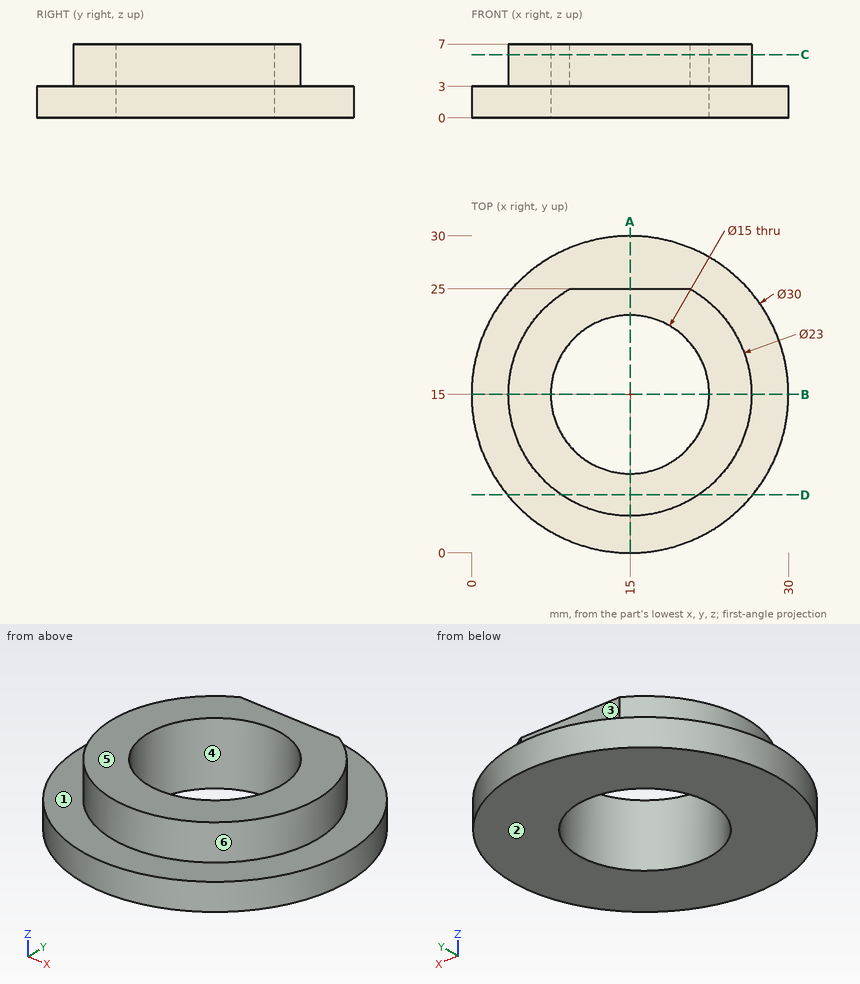
Check sheet for the drawn part. Datum: minimum x, y, z corner. Units: mm. A direction names the side the tool comes from. Coordinates: 2 decimals unless noted, no trailing zeros. Write each loop counter-clockwise with the first axis right and the second up, starting at its lowest first coordinate (ties: lowest second). Pieces come first, ordered by that corner, then holes. Notation, with made-up numbers: M -22,46 L 19,46 A16 cw 19,51 Z; hole C 58,-35 d1. An arc over 180 degrees is marked long. Use a Markdown table: item, result.
Q1. Thickness scan on line 1 (X direction, y = 17, z = 2); line 2 (Z direction, x = 22.5, y = 6.25); line 3 (X direction, y = 12.5, z = 6). Record the ranges inside material, lowest first.
Reply:
| item | result |
|---|---|
| line 1 | x = 0.13 to 7.77, 22.23 to 29.87 |
| line 2 | z = 0 to 3 |
| line 3 | x = 3.78 to 7.93, 22.07 to 26.22 |
Q2. Draft check along X on the marked faces 4, 5 and 6. Enter one of: +X half, -X half, draft (parallel to the pull), parting line (faces both ways), or undercut.
Reply:
| item | result |
|---|---|
| face 4 | undercut |
| face 5 | draft |
| face 6 | parting line |
Q3. Set-up check for the marked faces 1, 2 and 3: record each of +Z, -Z, +X, -X, +Y, -Y from which the full face is reachable in a straight line by a thin tool's end or side.
Reply:
| item | result |
|---|---|
| face 1 | +Z |
| face 2 | -Z, +X, -X, +Y, -Y |
| face 3 | +Z, +X, -X, +Y |
Q4. Go/stop test with flat-tipped pins: P1, Ø3, axis at x = 6.5, z = 2, coming from the -Y side; P2, Ø2, axis at y = 7, z = 5, coming from the -X side; P3, Ø2, axis at y = 22.5, z = 1, coming from the +X side. Record where each tip stops, or that it passes through.
Reply:
| item | result |
|---|---|
| P1 | stops at y = 1.73 |
| P2 | stops at x = 5.88 |
| P3 | stops at x = 28.52 |
Q5. Sectioned sample at D-D, the plane y = 5.5. Record the boundary of the cut face in (x, z).
Reply:
| item | result |
|---|---|
| outline | M 3.39,0 L 26.61,0 L 26.61,3 L 21.48,3 L 21.48,7 L 8.52,7 L 8.52,3 L 3.39,3 Z |
Q6. Sectioned sample at C-C, the plane z = 6. Record the boundary of the cut face in (x, y), plus the area to 3 significant figures.
Reply:
| item | result |
|---|---|
| outline | M 9.32,25 A11.5 ccw long 20.68,25 Z; hole C 15,15 d15 |
| area | 227 mm² |
Q7. Sectioned sample at B-B, the plane y = 15. Record the boundary of the cut face in (x, z), plus the area to 3 significant figures.
Reply:
| item | result |
|---|---|
| outline | M 0,0 L 7.5,0 L 7.5,7 L 3.5,7 L 3.5,3 L 0,3 Z; M 22.5,0 L 30,0 L 30,3 L 26.5,3 L 26.5,7 L 22.5,7 Z |
| area | 77.0 mm² |
Q8. Sectioned sample at A-A, the plane x = 15. Record the boundary of the cut face in (y, z), plus the area to 3 significant figures.
Reply:
| item | result |
|---|---|
| outline | M 0,0 L 7.5,0 L 7.5,7 L 3.5,7 L 3.5,3 L 0,3 Z; M 22.5,0 L 30,0 L 30,3 L 25,3 L 25,7 L 22.5,7 Z |
| area | 71.0 mm² |
